Geometry: final body of the model. Coordinates: model frame, mm. A direction names the side the tool comes from. Coordinates: 2 decimals unless noted, no trailing zeros. Loops run counter-clockwise (first coordinate to the right, second up) from the corner with the lowest first, then second, coordinate; pieces in that order, holes last. Notation, with made-up numbers: M -3,-5.5 L 12,-5.5 A16 cw 12,-1.5 Z; hole C -11,80 d9. An arc over 180 degrees is marked long. Write item = value, one per line. Start each with the question number.
```python
from build123d import *

# Parameters (mm, degrees)
BOSS_EXTRUDE1_DEPTH = 6
SKETCH2_R           = 2.5
BOSS_EXTRUDE2_DEPTH = 6
SKETCH3_R           = 4
BOSS_EXTRUDE3_DEPTH = 2
SKETCH4_R           = 3
BOSS_EXTRUDE4_DEPTH = 66
CHAMFER1_SIZE       = 0.5
SKETCH5_W           = 5
SKETCH5_H           = 36
CHAMFER2_SIZE       = 0.5


with BuildPart() as part:
    # Sketch1 → Boss-Extrude1 (new body)
    with BuildSketch(Plane.XY):
        Polygon((5.773502692, 0), (2.886751346, 5), (-2.886751346, 5), (-5.773502692, 0), (-2.886751346, -5), (2.886751346, -5), align=None)
    extrude(amount=BOSS_EXTRUDE1_DEPTH)

    # Sketch2 → Boss-Extrude2 (add)
    with BuildSketch(Plane(origin=(0, 0, 0), x_dir=(-1, 0, 0), z_dir=(0, 0, -1))):
        with Locations(Location((0, 0, 0), (0, 0, 180))):
            Circle(SKETCH2_R)
    extrude(amount=BOSS_EXTRUDE2_DEPTH)

    # Sketch3 → Boss-Extrude3 (add)
    with BuildSketch(Plane.XY.offset(6)):
        Circle(SKETCH3_R)
    extrude(amount=BOSS_EXTRUDE3_DEPTH)

    # Sketch4 → Boss-Extrude4 (add)
    with BuildSketch(Plane.XY.offset(8)):
        Circle(SKETCH4_R)
    extrude(amount=BOSS_EXTRUDE4_DEPTH)

    # Chamfer1
    chamfer1_edges = [part.edges().sort_by_distance(p)[0] for p in [
        (-3, 0, 74),
    ]]
    chamfer(chamfer1_edges, length=CHAMFER1_SIZE)

    # Sketch5 → Cut-Revolve1 (revolve, cut)
    with BuildSketch(Plane(origin=(0, 0, 0), x_dir=(1, 0, 0), z_dir=(0, 1, 0))):
        with Locations((5.25, -41)):
            Rectangle(SKETCH5_W, SKETCH5_H)
    revolve(axis=Axis((0, 0, 73.5), (0, 0, -1)), mode=Mode.SUBTRACT)

    # Chamfer2
    chamfer2_edges = [part.edges().sort_by_distance(p)[0] for p in [
        (-2.5, 0, -6),
    ]]
    chamfer(chamfer2_edges, length=CHAMFER2_SIZE)


solid = part.part
```
Item 1: Section query A-A (x = 0). Return the cut outline in (y, z).
Item 2: First-contact query: pin 1 (1.5 mm diameter, centred on y = 1, z = 45.5, fed in from +X); pin 2 (1.5 mm diameter, centred on x = 0, z = 12.5, fed in from +Y); pin 3 (2 mm diameter, centred on x = 0.5, y = 3, fed in from -Z). Flat tips, straight axial feed; report the tip coordinate or a pass-through.
Item 3: Pull-direction query (Z, two-part tool) for faces 3 (the cylindrical face through (-2.5, -0.1, -2.7)), 4 (the flat face through (2.5, 1.2, 0)), 5 (the flat face through (0, 0, 74)), 6 (the cylindrical face through (-0.596, 2.685, 40.748)); classes: released by +Z, released by -Z, zero draft, split by the parting line, or undercut.
Item 4: Line query: line 1 (Z direction, x = -2.25, y = 2.5); line 2 (Z direction, x = -0.25, y = -4.5); line 3 (Y direction, x = 0.25, z = 63). Output: solid intervals per line, ascending. Write a range as from..to.
Item 5: Reachability of faces 1 (the cylindrical face through (-3, 0, 66)), 2 (the flat face through (-4.35, -2.465, 2.958)) from +Z, -Z, +X, -X, +Y, -Y: full face, straight path, thin tool, end or side. Return the list, or none.
Item 6: Section query B-B (z = 64.5). Return the cut outline in (x, y).
Item 7: Section query C-C (z = 36). Return the cut outline in (x, y), plus the area to 3 significant figures.
Verdict:
q1.outline = M -5,0 L -2.5,0 L -2.5,-5.5 L -2,-6 L 2,-6 L 2.5,-5.5 L 2.5,0 L 5,0 L 5,6 L 4,6 L 4,8 L 3,8 L 3,23 L 2.75,23 L 2.75,59 L 3,59 L 3,73.5 L 2.5,74 L -2.5,74 L -3,73.5 L -3,59 L -2.75,59 L -2.75,23 L -3,23 L -3,8 L -4,8 L -4,6 L -5,6 Z
q2.pin_1 = 2.74
q2.pin_2 = 3
q2.pin_3 = -5.96
q3.face_3 = zero draft
q3.face_4 = released by -Z
q3.face_5 = released by +Z
q3.face_6 = undercut
q4.line_1 = 0..8
q4.line_2 = 0..6
q4.line_3 = -2.99..2.99
q5.face_1 = +Z
q5.face_2 = +Z, -Z, -X, -Y
q6.outline = C 0,0 d6
q7.outline = C 0,0 d5.5
q7.area = 23.8 mm2
